from build123d import *

# Parameters (mm, degrees)
SKETCH_1_W                = 80
SKETCH_1_H                = 235
EXTRUDE_1_DEPTH           = 10
SKETCH_20_W               = 82
SKETCH_20_H               = 14.219263271
CUT_EXTRUDE_3_DEPTH       = 2
HOLE_WIZARD_4_D           = 4.3
HOLE_WIZARD_4_CBORE_D     = 8
HOLE_WIZARD_4_CBORE_DEPTH = 5
SKETCH_26_W               = 13
SKETCH_26_H               = 87.5
EXTRUDE_3_DEPTH           = 10
FILLET_5_R                = 5
HOLE_WIZARD_1_D           = 5.4
HOLE_WIZARD_1_CBORE_D     = 10
HOLE_WIZARD_1_CBORE_DEPTH = 6
PATTERN_LINEAR_2_COUNT    = 2
PATTERN_LINEAR_2_PITCH    = 17.5
MOVE_FACE_1_BY            = 13
MOVE_FACE_1_2_BY          = 13
SKETCH_30_W               = 265.385639797
SKETCH_30_H               = 12.1
CUT_EXTRUDE_7_DEPTH       = 1.5
SKETCH_31_W               = 11.95
SKETCH_31_H               = 17.539728067
SKETCH_31_H_2             = 20.784895231
EXTRUDE_4_DEPTH           = 10
SKETCH_32_R               = 2
CUT_EXTRUDE_8_DEPTH       = 2
MM_1_D                    = 5
MM_1_DEPTH                = 10.1
MM_1_TIP                  = 1.502151548
FILLET_6_R                = 10
HOLE_WIZARD_M6_1_D        = 5
HOLE_WIZARD_M6_1_DEPTH    = 15
HOLE_WIZARD_M6_1_TIP      = 1.502151548
HOLE_WIZARD_M6_2_D        = 5
HOLE_WIZARD_M6_2_DEPTH    = 15
HOLE_WIZARD_M6_2_TIP      = 1.502151548
HOLE_WIZARD_M6_3_D        = 5
HOLE_WIZARD_M6_4_D        = 5


with BuildPart() as part:
    # 草图1 → 凸台-拉伸1 (new body)
    with BuildSketch(Plane.XY):
        with Locations((0, -117.5)):
            Rectangle(SKETCH_1_W, SKETCH_1_H)
    extrude(amount=EXTRUDE_1_DEPTH)

    # 草图20 → 切除-拉伸3 (cut)
    with BuildSketch(Plane.XY.offset(10)):
        with Locations((0, -232.009631635)):
            Rectangle(SKETCH_20_W, SKETCH_20_H)
    extrude(amount=-CUT_EXTRUDE_3_DEPTH, mode=Mode.SUBTRACT)

    # 打孔尺寸(%根据)开槽圆柱头螺钉的类型4 (through all)
    with Locations(Plane(origin=(0, 0, 0), x_dir=(-1, 0, 0), z_dir=(0, 0, -1))):
        with Locations((-22.5, -230), (22.5, -230)):
            CounterBoreHole(HOLE_WIZARD_4_D / 2, HOLE_WIZARD_4_CBORE_D / 2, HOLE_WIZARD_4_CBORE_DEPTH)

    # 草图26 → 凸台-拉伸3 (add)
    with BuildSketch(Plane.XY.offset(10)):
        with Locations((46.5, -43.75)):
            Rectangle(SKETCH_26_W, SKETCH_26_H)
    extrude_3 = extrude(amount=-EXTRUDE_3_DEPTH)

    # 镜向1: 凸台-拉伸3 across plane
    add(extrude_3.mirror(Plane(origin=(0, 0, 0), x_dir=(0, 0, 1), z_dir=(1, 0, 0))))

    # 圆角5
    fillet_5_edges = [part.edges().sort_by_distance(p)[0] for p in [
        (53, 0, 5),
        (-53, 0, 5),
    ]]
    fillet(fillet_5_edges, radius=FILLET_5_R)

    # 打孔尺寸(%根据)内六角圆柱头螺钉的类型1 (through all)
    with Locations(Plane.XY.offset(10)):
        with Locations((-47, -17.5), (-47, -52.5), (47, -52.5), (47, -17.5)):
            hole_wizard_1 = CounterBoreHole(HOLE_WIZARD_1_D / 2, HOLE_WIZARD_1_CBORE_D / 2, HOLE_WIZARD_1_CBORE_DEPTH)

    # 阵列(线性)2: 打孔尺寸(%根据)内六角圆柱头螺钉的类型1 ×2
    with Locations(*[(0, -i * PATTERN_LINEAR_2_PITCH, 0) for i in range(1, PATTERN_LINEAR_2_COUNT)]):
        add(hole_wizard_1, mode=Mode.SUBTRACT)

    # Move Face 1: a face moved outward by 13.0
    extrude(part.faces().sort_by_distance((40, -160.296095683, 4.94445972))[0], amount=MOVE_FACE_1_BY, dir=(1, 0, 0))

    # Move Face 1 2: a face moved outward by 13.0
    extrude(part.faces().sort_by_distance((-40, -160.296095683, 4.94445972))[0], amount=MOVE_FACE_1_2_BY, dir=(-1, 0, 0))

    # 草图30 → 切除-拉伸7 (cut)
    with BuildSketch(Plane.XY.offset(10)):
        with Locations((-68.564117246, -106)):
            Rectangle(SKETCH_30_W, SKETCH_30_H)
    extrude(amount=-CUT_EXTRUDE_7_DEPTH, mode=Mode.SUBTRACT)

    # 草图31 → 凸台-拉伸4 (add)
    with BuildSketch(Plane.XY.offset(10)):
        with Locations((-47.025, -226.230135967)):
            Rectangle(SKETCH_31_W, SKETCH_31_H)
        with Locations((47.025, -224.607552385)):
            Rectangle(SKETCH_31_W, SKETCH_31_H_2)
    extrude(amount=-EXTRUDE_4_DEPTH)

    # 草图32 → 切除-拉伸8 (cut)
    with BuildSketch(Plane.XY.offset(10)):
        with Locations((-41.05, -224.9)):
            Circle(SKETCH_32_R)
        with Locations((41.05, -224.9)):
            Circle(SKETCH_32_R)
    extrude(amount=-CUT_EXTRUDE_8_DEPTH, mode=Mode.SUBTRACT)

    # 大小mm 暗销孔1
    with Locations(Plane(origin=(0, 0, 0), x_dir=(-1, 0, 0), z_dir=(0, 0, -1))):
        with Locations((-32.5, -230), (32.5, -230)):
            Hole(MM_1_D / 2, depth=MM_1_DEPTH)
            with Locations((0, 0, -(MM_1_DEPTH + MM_1_TIP / 2))):  # 118° drill point
                Cone(0, MM_1_D / 2, MM_1_TIP, mode=Mode.SUBTRACT)

    # 圆角6
    fillet_6_edges = [part.edges().sort_by_distance(p)[0] for p in [
        (53, -235, 5),
        (-53, -235, 5),
    ]]
    fillet(fillet_6_edges, radius=FILLET_6_R)

    # M6 螺纹孔1
    with Locations(Plane.XY.offset(10)):
        with Locations((-41.5, -106), (41.5, -106)):
            Hole(HOLE_WIZARD_M6_1_D / 2, depth=HOLE_WIZARD_M6_1_DEPTH)
            with Locations((0, 0, -(HOLE_WIZARD_M6_1_DEPTH + HOLE_WIZARD_M6_1_TIP / 2))):  # 118° drill point
                Cone(0, HOLE_WIZARD_M6_1_D / 2, HOLE_WIZARD_M6_1_TIP, mode=Mode.SUBTRACT)

    # M6 螺纹孔2
    with Locations(Plane.XY.offset(10)):
        with Locations((0, -208)):
            Hole(HOLE_WIZARD_M6_2_D / 2, depth=HOLE_WIZARD_M6_2_DEPTH)
            with Locations((0, 0, -(HOLE_WIZARD_M6_2_DEPTH + HOLE_WIZARD_M6_2_TIP / 2))):  # 118° drill point
                Cone(0, HOLE_WIZARD_M6_2_D / 2, HOLE_WIZARD_M6_2_TIP, mode=Mode.SUBTRACT)

    # M6 螺纹孔3 (through all)
    with Locations(Plane.XY.offset(10)):
        with Locations((0, -155), (0, -182)):
            Hole(HOLE_WIZARD_M6_3_D / 2)

    # M6 螺纹孔4 (through all)
    with Locations(Plane.XY.offset(10)):
        with Locations((0, -129)):
            Hole(HOLE_WIZARD_M6_4_D / 2)


solid = part.part
Can you work these out from the model? Positions are in its coordinate system, mm. A direction names the side the tool comes from. Coordinates: 2 decimals unless noted, no trailing zeros. Write each loop counter-clockwise with the first axis right and the second up, starting at its lowest first coordinate (ties: lowest second). Pieces come first, ordered by that corner, then holes. Notation, with made-up numbers: (-4.5, 11.25) -> (41.5, 11.25) arc R21 cw to (41.5, 36.25) -> close; hole circle Ø2 at (-33.5, 88.5). An arc over 180 degrees is marked (long way). Answer as CSV lines item,"result".
1) On a 3-axis mill with a long thin cutter (end or side, diameter ignored), from which of +Z, -Z, +X, -X, +Y, -Y can I reach the whole of each face in a straight line? I mean faces 4 (the flat face through (53, -117, 5)), 5 (the cylindrical face through (-24.65, -226.627, 2.465)), 6 (the cylindrical face through (43, -67, 7)). Say none if no direction works.
Check result:
face 4,"+Z, -Z, +X, +Y, -Y"
face 5,"-Z"
face 6,"+Z"
2) If we section it at A-A on x = -22.5: Please give me the cut outline in (y, z).
Check result:
outline,"(-235, 0) -> (-234, 0) -> (-234, 5) -> (-232.15, 5) -> (-232.15, 8) -> (-235, 8) -> close; (-227.85, 5) -> (-226, 5) -> (-226, 0) -> (0, 0) -> (0, 10) -> (-99.95, 10) -> (-99.95, 8.5) -> (-112.05, 8.5) -> (-112.05, 10) -> (-224.9, 10) -> (-224.9, 8) -> (-227.85, 8) -> close"
3) If we mould it in two halves opening along Y, with no side actions, what happens to faces 1 (the cylindrical face through (44.425, -16.689, 1.972)), 2 (the flat face through (-1, -235, 4)), 3 (the flat face through (1, 0, 5))? For each: +Y half, -Y half, draft (parallel to the pull), parting line (faces both ways), or undercut.
Check result:
face 1,"undercut"
face 2,"-Y half"
face 3,"+Y half"
4) If I drill on line 1 (Y direction, x = 0, z = 5.25); line 2 (Y direction, x = -32.5, z = 5); line 3 (Y direction, x = 2, z = 9.5), over which ranges is the centre line in solid material (lowest first)? Write a range as from..to.
Check result:
line 1,"-235..-210.5, -205.5..-184.5, -179.5..-157.5, -152.5..-131.5, -126.5..0"
line 2,"-235..-232.5, -227.5..0"
line 3,"-224.9..-209.5, -206.5..-183.5, -180.5..-156.5, -153.5..-130.5, -127.5..-112.05, -99.95..0"
5) If we section it at B-B on z = 2.25: Count the separate pieces of the cut face and the enclosed holes in it, then the cut area to 3 significant figures.
Check result:
separate pieces,"1"
enclosed holes,"18"
area,"24,400 mm²"
6) Will these pins go through, and if not, where does the flat tip stop? P1, Ø5, axis at x = -22.5, y = -230, coming from the +Z side; P2, Ø11, axis at x = 46.5, y = -19.5, coming from the +Z side; P3, Ø7, axis at x = -47, y = -17.5, coming from the +Z side; P4, Ø2, axis at y = -232.5, z = 9, coming from the -X side.
Check result:
P1,"z = 8"
P2,"z = 10"
P3,"z = 4"
P4,"x = -50.6"
7) If we section it at D-D on x = 0: Please give me the cut outline in (y, z).
Check result:
outline,"(-235, 0) -> (-210.5, 0) -> (-210.5, 10) -> (-224.9, 10) -> (-224.9, 8) -> (-235, 8) -> close; (-205.5, 0) -> (-184.5, 0) -> (-184.5, 10) -> (-205.5, 10) -> close; (-179.5, 0) -> (-157.5, 0) -> (-157.5, 10) -> (-179.5, 10) -> close; (-152.5, 0) -> (-131.5, 0) -> (-131.5, 10) -> (-152.5, 10) -> close; (-126.5, 0) -> (0, 0) -> (0, 10) -> (-99.95, 10) -> (-99.95, 8.5) -> (-112.05, 8.5) -> (-112.05, 10) -> (-126.5, 10) -> close"
8) If we section it at C-C on y = -106: Please give me the cut outline in (x, z).
Check result:
outline,"(-53, 0) -> (-44, 0) -> (-44, 8.5) -> (-53, 8.5) -> close; (-39, 0) -> (39, 0) -> (39, 8.5) -> (-39, 8.5) -> close; (44, 0) -> (53, 0) -> (53, 8.5) -> (44, 8.5) -> close"
